Work out the finished part from the listing and answer in its coordinate system (mm). A direction names the side the tool comes from. Round coordinates to 2 decimals unless told otherwise and drop trailing zeros. Write each loop counter-clockwise with the first axis right and the second up, starting at its lowest first coordinate (ties: lowest second). Pieces come first, ordered by that corner, then holes. Notation, with made-up numbers: M 67.25,40.5 L 95.25,40.5 A9 cw 95.25,52.5 Z; hole C -13,14 d6. An arc over 180 degrees is marked long. One line per item, written item: value. Start each with the question number.
Q1. Given pin 1 Ø3.5 at (x, y) = (10, 0) entering from +Z; pin 2 Ø8 at (y, z) = (9.5, 9) entering from +X; pin 3 Ø3 at (x, z) = (15, 5) entering from +Y; pin 4 Ø5 at (x, y) = (0, 0) entering from +Z, each flat-ended and moving along its own axis, determine where each tip first touches the part or whether it passes through.
Q2. Find section D-D (y = 10). Write down the section's boundary in (x, z), and give its area (3 significant figures).
Q3. The mould has two halves that part along X. Classify faces 1 (the flat face through (0, -5, 0)), 2 (the cylindrical face through (12.932, -5.362, 7.451)), 3 (the flat face through (-7, -7, 1)): released by +X, released by -X, zero draft, split by the parting line, or undercut.
Q4. Consider probe 1 along Y at (x, z) = (0, 3); probe 2 along X at (y, z) = (-7.5, 9); probe 3 along Z at (x, y) = (10.5, 9.5). Determine where each line is inside the solid, lowest interval first.
Q5. A tool of negligible diameter and unlimited length cuts with its end or side. For faces 4 (the cylindrical face through (-20.9, -11.8, 2)), 5 (the flat face through (0, 10, 1)), from which of +Z, -Z, +X, -X, +Y, -Y can it reach the whole face along a straight path? Write none if from no direction.
Q6. Find section C-C (z = 6). Count the separate pieces of the cut face and the enclosed holes in it, and give its area (3 significant figures).
Q7. Find section A-A (x = 0). Write down the section's boundary in (y, z).
Q8. Find section B-B (y = 0). Write down the section's boundary in (x, z), and give its area (3 significant figures).
from build123d import *

# Parameters (mm, degrees)
FLANGE_DISC_SKETCH_R    = 24
FLANGE_DISC_48_DEPTH    = 4
HUB_SKETCH_R            = 14
HUB_28_DEPTH            = 7
FLANGE_HOLES_SKETCH_R   = 1.5
FLANGE_HOLES_3X_3_DEPTH = 10
HUB_HOLES_SKETCH_R      = 2
HUB_HOLES_8X_4_DEPTH    = 10
CENTRE_SPIGOT_SKETCH_R  = 4
CENTRE_SPIGOT_8_DEPTH   = 5
BORE_SKETCH_R           = 3
BORE_6_DEPTH            = 30
EDGE_START              = -30
EDGE_NOTCHES_DEPTH      = 30


with BuildPart() as part:
    # Flange Disc Sketch → Flange Disc Ø48 (new body)
    with BuildSketch(Plane.XY):
        Circle(FLANGE_DISC_SKETCH_R)
    extrude(amount=FLANGE_DISC_48_DEPTH)

    # Hub Sketch → Hub Ø28 (add)
    with BuildSketch(Plane.XY.offset(4)):
        Circle(HUB_SKETCH_R)
    extrude(amount=HUB_28_DEPTH)

    # Flange Holes Sketch → Flange Holes 3xØ3 (cut)
    with BuildSketch(Plane.XY.offset(4)):
        with Locations((0, 18)):
            Circle(FLANGE_HOLES_SKETCH_R)
        with Locations((15.588457268, -9)):
            Circle(FLANGE_HOLES_SKETCH_R)
        with Locations((-15.588457268, -9)):
            Circle(FLANGE_HOLES_SKETCH_R)
    extrude(amount=-FLANGE_HOLES_3X_3_DEPTH, mode=Mode.SUBTRACT)

    # Hub Holes Sketch → Hub Holes 8xØ4 (cut)
    with BuildSketch(Plane.XY.offset(11)):
        with Locations((0, 10)):
            Circle(HUB_HOLES_SKETCH_R)
        with Locations((7.071067812, 7.071067812)):
            Circle(HUB_HOLES_SKETCH_R)
        with Locations((10, 0)):
            Circle(HUB_HOLES_SKETCH_R)
        with Locations((7.071067812, -7.071067812)):
            Circle(HUB_HOLES_SKETCH_R)
        with Locations((0, -10)):
            Circle(HUB_HOLES_SKETCH_R)
        with Locations((-7.071067812, -7.071067812)):
            Circle(HUB_HOLES_SKETCH_R)
        with Locations((-10, 0)):
            Circle(HUB_HOLES_SKETCH_R)
        with Locations((-7.071067812, 7.071067812)):
            Circle(HUB_HOLES_SKETCH_R)
    extrude(amount=-HUB_HOLES_8X_4_DEPTH, mode=Mode.SUBTRACT)

    # Centre Spigot Sketch → Centre Spigot Ø8 (add)
    with BuildSketch(Plane.XY.offset(11)):
        Circle(CENTRE_SPIGOT_SKETCH_R)
    extrude(amount=CENTRE_SPIGOT_8_DEPTH)

    # Bore Sketch → Bore Ø6 (cut)
    with BuildSketch(Plane.XY.offset(16)):
        Circle(BORE_SKETCH_R)
    extrude(amount=-BORE_6_DEPTH, mode=Mode.SUBTRACT)

    # Edge Notches Sketch → Edge Notches (cut)
    with BuildSketch(Plane.XY.offset(4).offset(EDGE_START)):
        with BuildLine():
            ThreePointArc((-17.92809871, 15.955665973), (-20.784609691, 12), (-22.782061422, 7.548355939))
            Line((-22.782061422, 7.548355939), (-16.571312466, 6.046586076))
            ThreePointArc((-16.571312466, 6.046586076), (-15.276688123, 8.82), (-13.52215338, 11.327884531))
            Line((-13.52215338, 11.327884531), (-17.92809871, 15.955665973))
        make_face()
        with BuildLine():
            ThreePointArc((-13.52215338, 11.327884531), (-15.276688123, 8.82), (-16.571312466, 6.046586076))
            Line((-16.571312466, 6.046586076), (-15.98177362, 5.904034561))
            ThreePointArc((-15.98177362, 5.904034561), (-12.678611911, 7.32), (-13.103930725, 10.888604672))
            Line((-13.103930725, 10.888604672), (-13.52215338, 11.327884531))
        make_face()
        with BuildLine():
            Line((16.571312466, 6.046586076), (22.782061422, 7.548355939))
            ThreePointArc((22.782061422, 7.548355939), (20.784609691, 12), (17.92809871, 15.955665973))
            Line((17.92809871, 15.955665973), (13.52215338, 11.327884531))
            ThreePointArc((13.52215338, 11.327884531), (15.276688123, 8.82), (16.571312466, 6.046586076))
        make_face()
        with BuildLine():
            ThreePointArc((16.571312466, 6.046586076), (15.276688123, 8.82), (13.52215338, 11.327884531))
            Line((13.52215338, 11.327884531), (13.103930725, 10.888604672))
            ThreePointArc((13.103930725, 10.888604672), (12.678611911, 7.32), (15.98177362, 5.904034561))
            Line((15.98177362, 5.904034561), (16.571312466, 6.046586076))
        make_face()
        with BuildLine():
            Line((-3.049159085, -17.374470607), (-4.853962711, -23.504021911))
            ThreePointArc((-4.853962711, -23.504021911), (0, -24), (4.853962711, -23.504021911))
            Line((4.853962711, -23.504021911), (3.049159085, -17.374470607))
            ThreePointArc((3.049159085, -17.374470607), (0, -17.64), (-3.049159085, -17.374470607))
        make_face()
        with BuildLine():
            Line((-2.877842895, -16.792639233), (-3.049159085, -17.374470607))
            ThreePointArc((-3.049159085, -17.374470607), (0, -17.64), (3.049159085, -17.374470607))
            Line((3.049159085, -17.374470607), (2.877842895, -16.792639233))
            ThreePointArc((2.877842895, -16.792639233), (0, -14.64), (-2.877842895, -16.792639233))
        make_face()
    extrude(amount=EDGE_NOTCHES_DEPTH, mode=Mode.SUBTRACT)


solid = part.part
The answers:
1. pin 1: z = 1
1. pin 2: x = 12.87
1. pin 3: y = 19.58
1. pin 4: through
2. outline: M -12.52,0 L 12.52,0 L 12.52,4 L 9.8,4 L 9.8,11 L 2,11 L 2,1 L -2,1 L -2,11 L -9.8,11 L -9.8,4 L -12.52,4 Z
2. area: 197 mm2
3. face 1: zero draft
3. face 2: split by the parting line
3. face 3: undercut
4. probe 1: -14.64 to -12, -8 to -3, 3 to 8, 12 to 16.5, 19.5 to 24
4. probe 2: -11.82 to -9.02, -5.12 to 5.12, 9.02 to 11.82
4. probe 3: 0 to 4
5. face 4: +Z, -Z, -X
5. face 5: +Z
6. separate pieces: 1
6. enclosed holes: 9
6. area: 487 mm2
7. outline: M -14.64,0 L -3,0 L -3,16 L -4,16 L -4,11 L -8,11 L -8,1 L -12,1 L -12,11 L -14,11 L -14,4 L -14.64,4 Z; M 3,0 L 16.5,0 L 16.5,4 L 14,4 L 14,11 L 12,11 L 12,1 L 8,1 L 8,11 L 4,11 L 4,16 L 3,16 Z; M 19.5,0 L 24,0 L 24,4 L 19.5,4 Z
8. outline: M -24,0 L -3,0 L -3,16 L -4,16 L -4,11 L -8,11 L -8,1 L -12,1 L -12,11 L -14,11 L -14,4 L -24,4 Z; M 3,0 L 24,0 L 24,4 L 14,4 L 14,11 L 12,11 L 12,1 L 8,1 L 8,11 L 4,11 L 4,16 L 3,16 Z
8. area: 252 mm2
